from build123d import *

# Parameters (mm, degrees)
CHAMFER1_SIZE      = 2
SKETCH2_R          = 4
CUT_EXTRUDE1_DEPTH = 49
SKETCH3_R          = 7
CUT_EXTRUDE2_DEPTH = 6


with BuildPart() as part:
    # Sketch1 → Revolve1 (revolve)
    with BuildSketch(Plane.XY, mode=Mode.PRIVATE) as revolve1_sk:
        Polygon((-28.741506647, 6), (-28.741506647, 51.5), (-21.741506647, 51.5), (-21.741506647, 70.5), (-2.741506647, 70.5), (-2.741506647, 19.745937962), (-10.031019202, 14.747415066), (-10.031019202, 6), align=None)
    revolve(revolve1_sk.sketch.rotate(Axis((-75.394387001, 0, 0), (1, 0, 0)), 90), axis=Axis((-75.394387001, 0, 0), (1, 0, 0)))

    # Chamfer1
    chamfer1_edges = [part.edges().sort_by_distance(p)[0] for p in [
        (-2.741506647, 0, -70.5),
    ]]
    chamfer(chamfer1_edges, length=CHAMFER1_SIZE)

    # Sketch2 → Cut-Extrude1 (cut)
    with BuildSketch(Plane(origin=(-2.741506647, 0, 0), x_dir=(0, 0, -1), z_dir=(1, 0, 0))):
        with Locations((0, -60.5)):
            Circle(SKETCH2_R)
        with Locations((-60.5, 0)):
            Circle(SKETCH2_R)
        with Locations((0, 60.5)):
            Circle(SKETCH2_R)
        with Locations((60.5, 0)):
            Circle(SKETCH2_R)
    extrude(amount=-CUT_EXTRUDE1_DEPTH, mode=Mode.SUBTRACT)

    # Sketch3 → Cut-Extrude2 (cut)
    with BuildSketch(Plane(origin=(-2.741506647, 0, 0), x_dir=(0, 0, -1), z_dir=(1, 0, 0))):
        with Locations((-60.5, 0)):
            Circle(SKETCH3_R)
        with Locations((0, 60.5)):
            Circle(SKETCH3_R)
        with Locations((60.5, 0)):
            Circle(SKETCH3_R)
        with Locations((0, -60.5)):
            Circle(SKETCH3_R)
    extrude(amount=-CUT_EXTRUDE2_DEPTH, mode=Mode.SUBTRACT)


solid = part.part
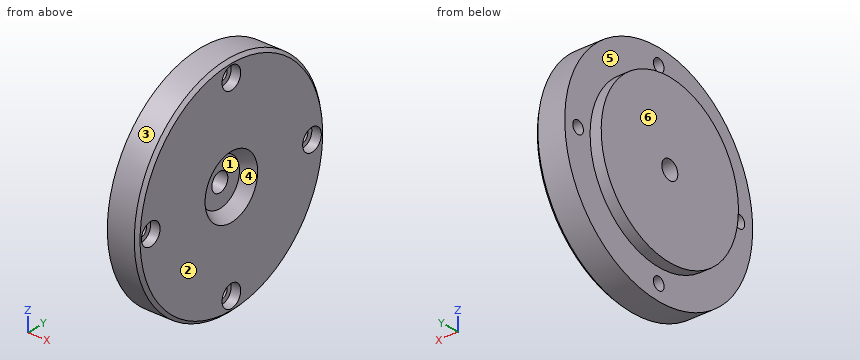
Read the model definition and answer for the solid it produces. Units are mm, in the model's axes. Face numbers are marked on the shaded views. A direction names the side the tool comes from. Round coordinates to 2 decimals unless told otherwise and drop trailing zeros. Order: outer loops, then holes, each group sorted by start corner. A loop starts at its lowest first (then second) coordinate and runs counter-clockwise, first axis right, second up. Notation, with made-up numbers: (-38, -8) - (1, -8) arc R22 ccw to (1, 12) - close; hole circle Ø10 at (36, 79.25). An arc over 180 degrees is marked (long way). Use one line per item in the form item = value. Start each with the question number.
(1) Determine the mould class of the marked faces 1, 2, 3 and 4 for opening direction Y: +Y half, -Y half, draft (parallel to the pull), parting line (faces both ways), or undercut.
(2) The part is cut by section C-C (x = -14). Give the vertices of the cut face in (y, z).
(3) For the marked faces 5 and 6, determine the directions among +Z, -Z, +X, -X, +Y, -Y from which every point of the face is accessible in a straight line to the end or side of a thin tool.
(4) Find the intervals of material crossed by line 1 along Z through (x, y) = (-12.5, -1); line 2 along X through (y, z) = (47, 42); line 3 along Y through (x, z) = (-6.6, 0), in increasing order. Write a range as from..to.
(5) The part is cut by section A-A (z = 0). Count the separate pieces of the cut face and the enclosed holes in it, then the cut area to 3 significant figures.
(6) Flat-ended cylindrical pins translate along their axes: pin 1 Ø11 at (y, z) = (0, 60.5) entering from -X; pin 2 Ø5 at (x, y) = (-18, 53.5) entering from +Z; pin 3 Ø1.5 at (x, y) = (-9, 25.5) entering from -Z. Find the tip coordinate at first contact, or state that the pin passes through.
(7) The part is cut by section D-D (x = -24). Give the vertices of the cut face in (y, z), then the cut area to 3 significant figures.
Checked values:
q1.face_1 = undercut
q1.face_2 = draft
q1.face_3 = parting line
q1.face_4 = undercut
q2.outline = circle Ø141 at (0, 0); hole circle Ø8 at (-60.5, 0); hole circle Ø12 at (0, 0); hole circle Ø8 at (0, -60.5); hole circle Ø8 at (0, 60.5); hole circle Ø8 at (60.5, 0)
q3.face_5 = -X
q3.face_6 = +Z, -Z, -X, +Y, -Y
q4.line_1 = -70.49..-64.37, -56.63..-5.92, 5.92..56.63, 64.37..70.49
q4.line_2 = -21.74..-2.74
q4.line_3 = -70.5..-67.5, -53.5..-17.1, 17.1..53.5, 67.5..70.5
q5.separate_pieces = 4
q5.enclosed_holes = 0
q5.area = 2,540 mm^2
q6.pin_1 = -21.74
q6.pin_2 = 48.67
q6.pin_3 = -66.01
q7.outline = circle Ø103 at (0, 0); hole circle Ø12 at (0, 0)
q7.area = 8,220 mm^2
